Input: part model. Units: mm. Frame: model coordinates. Face numbers are marked on the shaded views. Round coordinates to 2 decimals unless told otherwise and drop trailing zeros. Write each loop counter-clockwise with the first axis right and the second up, starting at its lowest first coordinate (ties: lowest second). Pieces come first, ordered by that corner, then holes. Notation, with made-up numbers: (-11.5, 84) - (-6.5, 84) arc R29 cw to (-6.5, 121) - close; hole circle Ø1 at (9, 28). An arc over 180 degrees is marked (long way). One line per item, written item: value. Start each with the question number.
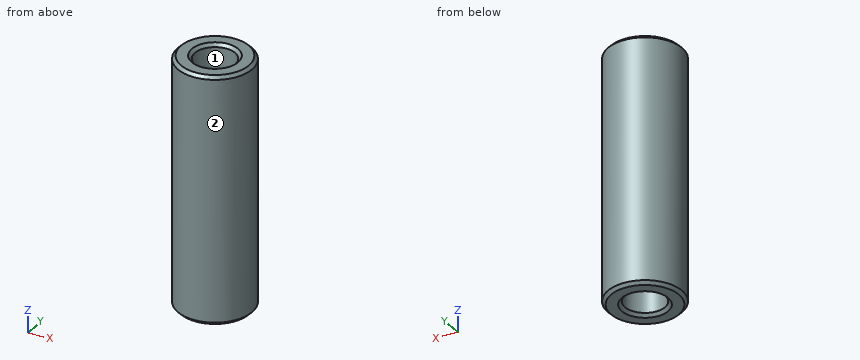
```python
from build123d import *


with BuildPart() as part:
    # Sketch2 → Revolve1 (revolve)
    with BuildSketch(Plane(origin=(0, 0, 0), x_dir=(1, 0, 0), z_dir=(0, 1, 0))):
        Polygon((1.5, 0), (2.2, 0), (2.4, 0.2), (2.4, 15.8), (2.2, 16), (1.5, 16), (1.3, 15.8), (1.3, 0.2), align=None)
    revolve(axis=Axis((0, 0, 0), (0, 0, -1)))


solid = part.part
```
Q1. Material intervals for probe 1 along Y at (x, z) = (0, -3.75); probe 2 along X at (y, z) = (-0.55, -10.75), sorted ascending. Write a range as from..to.
Q2. Contact query for flat-ended pins moving along their axis: pin 1 Ø1 at (y, z) = (1, -3) entering from -X; pin 2 Ø1 at (y, z) = (1.5, -3) entering from +X. Output: stop coordinate, or through.
Q3. Pull-direction query (Y, two-part tool) for the marked faces 1 and 2; classes: pulls with the +Y half, pulls with the -Y half, needs draft (parallel to the pull), parting line crosses it, or undercut.
Q4. Cut plane A-A, the plane y = 0. Output: boundary loops of the cut face in (x, z), and give its area (3 significant figures).
Q5. Cut plane C-C, the plane z = -6. Output: boundary loops of the cut face in (x, y), and give its area (3 significant figures).
A:
1. probe 1: y = -2.4..-1.3, 1.3..2.4
1. probe 2: x = -2.34..-1.18, 1.18..2.34
2. pin 1: stops at x = -2.35
2. pin 2: stops at x = 2.18
3. face 1: undercut
3. face 2: parting line crosses it
4. outline: (-2.4, -15.8) - (-2.2, -16) - (-1.5, -16) - (-1.3, -15.8) - (-1.3, -0.2) - (-1.5, 0) - (-2.2, 0) - (-2.4, -0.2) - close; (1.3, -15.8) - (1.5, -16) - (2.2, -16) - (2.4, -15.8) - (2.4, -0.2) - (2.2, 0) - (1.5, 0) - (1.3, -0.2) - close
4. area: 35.0 mm²
5. outline: circle Ø4.8 at (0, 0); hole circle Ø2.6 at (0, 0)
5. area: 12.8 mm²
